```python
from build123d import *

# Parameters (mm, degrees)
SKETCH_1_W                   = 50
SKETCH_1_H                   = 50
EXTRUDE_1_DEPTH              = 3
HOLE_WIZARD_M5_1_D           = 5.8
HOLE_WIZARD_M5_1_CSINK_D     = 11.2
HOLE_WIZARD_M5_1_CSINK_ANGLE = 90
CHAMFER_1_SIZE               = 2
SKETCH_8_R                   = 19.2
SKETCH_8_R_2                 = 16.8
CUT_EXTRUDE_2_DEPTH          = 1.5


with BuildPart() as part:
    # 草图1 → 凸台-拉伸1 (new, symmetric)
    with BuildSketch(Plane.XY):
        Rectangle(SKETCH_1_W, SKETCH_1_H)
    extrude(amount=EXTRUDE_1_DEPTH, both=True)

    # M5 六角凹锥坑螺钉的锥形沉头孔1 (through all)
    with Locations(Plane.XY.offset(3)):
        with Locations((-19, 19), (19, 19), (-19, -19), (19, -19)):
            CounterSinkHole(HOLE_WIZARD_M5_1_D / 2, HOLE_WIZARD_M5_1_CSINK_D / 2, counter_sink_angle=HOLE_WIZARD_M5_1_CSINK_ANGLE)

    # 倒角1
    chamfer_1_edges = [part.edges().sort_by_distance(p)[0] for p in [
        (25, -25, 0),
        (-25, -25, 0),
        (-25, 25, 0),
        (25, 25, 0),
    ]]
    chamfer(chamfer_1_edges, length=CHAMFER_1_SIZE)

    # 草图8 → 切除-拉伸2 (cut)
    with BuildSketch(Plane(origin=(0, 0, -3), x_dir=(-1, 0, 0), z_dir=(0, 0, -1))):
        Circle(SKETCH_8_R)
        Circle(SKETCH_8_R_2, mode=Mode.SUBTRACT)
    extrude(amount=-CUT_EXTRUDE_2_DEPTH, mode=Mode.SUBTRACT)


solid = part.part
```
Here's how the part is built. I have some questions about the finished solid (model axes, mm). Round coordinates to 2 decimals unless told otherwise and drop trailing zeros. Order: outer loops, then holes, each group sorted by start corner. A loop starts at its lowest first (then second) coordinate and runs counter-clockwise, first axis right, second up. Notation, with made-up numbers: M 49.25,-14 L 84.25,-14 A9 ccw 84.25,1 Z; hole C 28,60.5 d3. An arc over 180 degrees is marked long. One line per question, with ' | ' between items.
1) I want a section at A-A, the plane z = 1.7. Write out the boundary of the cut face in (x, y).
Working result:
outline: M -25,-23 L -23,-25 L 23,-25 L 25,-23 L 25,23 L 23,25 L -23,25 L -25,23 Z; hole C -19,-19 d8.6; hole C -19,19 d8.6; hole C 19,-19 d8.6; hole C 19,19 d8.6
2) I want a section at D-D, the plane x = 18. State how many separate pieces and enclosed holes the cut face has, then the cut area to 3 significant figures.
Working result:
separate pieces: 3 | enclosed holes: 0 | area: 199 mm²
3) I want a section at B-B, the plane x = 0. Write out the boundary of the cut face in (y, z), then the cut area to 3 significant figures.
Working result:
outline: M -25,-3 L -19.2,-3 L -19.2,-1.5 L -16.8,-1.5 L -16.8,-3 L 16.8,-3 L 16.8,-1.5 L 19.2,-1.5 L 19.2,-3 L 25,-3 L 25,3 L -25,3 Z | area: 293 mm²
4) I need wall thicknesses on line 1 along Y through (x, z) = (-19, -0.6); line 2 along Y through (x, z) = (6, -1.6). Which ranges of each line are inside material? Lowest first, please.
Working result:
line 1: -25 to -21.9, -16.1 to 16.1, 21.9 to 25 | line 2: -25 to -18.24, -15.69 to 15.69, 18.24 to 25
5) If we mould it in two halves opening along X, with no side actions, what happens to faces 1 (the face through (0, -17, -1.5)), 2 (the face through (-24, -24, 0)), 3 (the face through (25, 0, 0))? For each: +X half, -X half, draft (parallel to the pull), parting line (faces both ways), or undercut.
Working result:
face 1: undercut | face 2: -X half | face 3: +X half
6) For pin 1 Ø4.5 at (x, y) = (19, 19) entering from -Z; pin 2 Ø9.5 at (x, y) = (-19, 19) entering from -Z; pin 3 Ø7.5 at (x, y) = (-19, -19) entering from +Z, each with a flat end and sliding along its axis, tell me the tip position at first contact or that it passes through.
Working result:
pin 1: through | pin 2: z = -3 | pin 3: z = 1.15
